For this review, take the finished solid that the model builds, in its own axes (mm). Coordinates: 2 decimals unless noted, no trailing zeros. Write each loop counter-clockwise with the first axis right and the second up, starting at its lowest first coordinate (ties: lowest second). Pieces come first, ordered by that corner, then holes. Notation, with made-up numbers: (70.25, 4.25) -> (99.25, 4.25) arc R21 ccw to (99.25, 9.25) -> close; hole circle Ø3 at (-8.5, -22). An arc over 180 degrees is marked (long way). One line per item, written item: value. Start each with the question number.
1) Add section B-B (y = -111). State the section outline as (x, z) points.
2) For pin 1 Ø2.5 at (x, y) = (13, 111) entering from -Z, flat-tipped, find the tip position at first contact; note if it passes through.
3) Add section A-A (x = 13). State the section outline as (y, z) points, and give its area (3 significant figures).
4) For probe 1 along Y at (x, z) = (13, 1.5); probe 2 along Y at (x, z) = (-27, 2); probe 3 along Y at (x, z) = (32, 2.9), list the stretches that pass through material, from the lowest coordinate up. Write a range as from..to.
from build123d import *

# Parameters (mm, degrees)
SKETCH_1_W          = 80
SKETCH_1_H          = 243
EXTRUDE_1_DEPTH     = 3
SKETCH_4_R          = 2.2
CUT_EXTRUDE_2_DEPTH = 10
SKETCH_5_R          = 2.2
CUT_EXTRUDE_3_DEPTH = 10


with BuildPart() as part:
    # 草图1 → 凸台-拉伸1 (new body)
    with BuildSketch(Plane.XY):
        Rectangle(SKETCH_1_W, SKETCH_1_H)
    extrude(amount=EXTRUDE_1_DEPTH)

    # 草图4 → 切除-拉伸2 (cut)
    with BuildSketch(Plane(origin=(0, 0, 0), x_dir=(-1, 0, 0), z_dir=(0, 0, -1))):
        with Locations((-31, -68.5)):
            Circle(SKETCH_4_R)
        with Locations((-31, -93.5)):
            Circle(SKETCH_4_R)
    cut_extrude_2 = extrude(amount=-CUT_EXTRUDE_2_DEPTH, mode=Mode.SUBTRACT)

    # 镜向1: 切除-拉伸2 across plane
    add(cut_extrude_2.mirror(Plane.ZX), mode=Mode.SUBTRACT)

    # 草图5 → 切除-拉伸3 (cut)
    with BuildSketch(Plane(origin=(0, 0, 0), x_dir=(-1, 0, 0), z_dir=(0, 0, -1))):
        with Locations((-13, 111)):
            Circle(SKETCH_5_R)
        with Locations((-13, -111)):
            Circle(SKETCH_5_R)
        with Locations((27, 90)):
            Circle(SKETCH_5_R)
        with Locations((27, -90)):
            Circle(SKETCH_5_R)
    extrude(amount=-CUT_EXTRUDE_3_DEPTH, mode=Mode.SUBTRACT)


solid = part.part
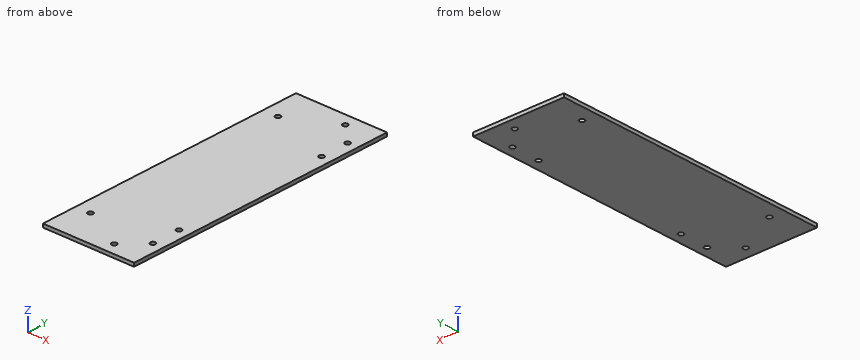
Numbers:
1. outline: (-40, 0) -> (10.8, 0) -> (10.8, 3) -> (-40, 3) -> close; (15.2, 0) -> (40, 0) -> (40, 3) -> (15.2, 3) -> close
2. pin 1: through
3. outline: (-121.5, 0) -> (-113.2, 0) -> (-113.2, 3) -> (-121.5, 3) -> close; (-108.8, 0) -> (108.8, 0) -> (108.8, 3) -> (-108.8, 3) -> close; (113.2, 0) -> (121.5, 0) -> (121.5, 3) -> (113.2, 3) -> close
3. area: 703 mm²
4. probe 1: -121.5..-113.2, -108.8..108.8, 113.2..121.5
4. probe 2: -121.5..-92.2, -87.8..87.8, 92.2..121.5
4. probe 3: -121.5..-95.46, -91.54..-70.46, -66.54..66.54, 70.46..91.54, 95.46..121.5
